Check sheet for the drawn part. Datum: minimum x, y, z corner. Units: mm. Give positions to 0.01 mm unless a question says otherwise; leave off trailing zeros. Order: outer loops, then holes, each group sorted by start corner. A loop starts at its lowest first (then second) coordinate and runs counter-clockwise, first axis right, second up. Notation, with made-up numbers: (15, 56.25) -> (53, 56.25) arc R13 cw to (53, 76.25) -> close; hole circle Ø3 at (-25.75, -28). An arc over 180 degrees is marked (long way). Return JSON: item names as keys, results as strings. Group by question number.
(1) Cross-section at A-A on z = 3.45. Enter the section's corners in (x, y).
(2) Cross-section at B-B on x = 15.25. Enter the section's corners in (y, z) (3 decimals), then the cut area to 3 significant figures.
(3) Cross-section at C-C on y = 95. Enter the section's corners in (x, z), then the cut area to 3 significant figures.
(4) Thickness scan on line 1 along X through (y, z) = (53.5, 3.8); line 2 along X through (y, z) = (51, 1.2); line 3 along Y through (x, z) = (3.25, 3.15). Record the ranges inside material, lowest first.
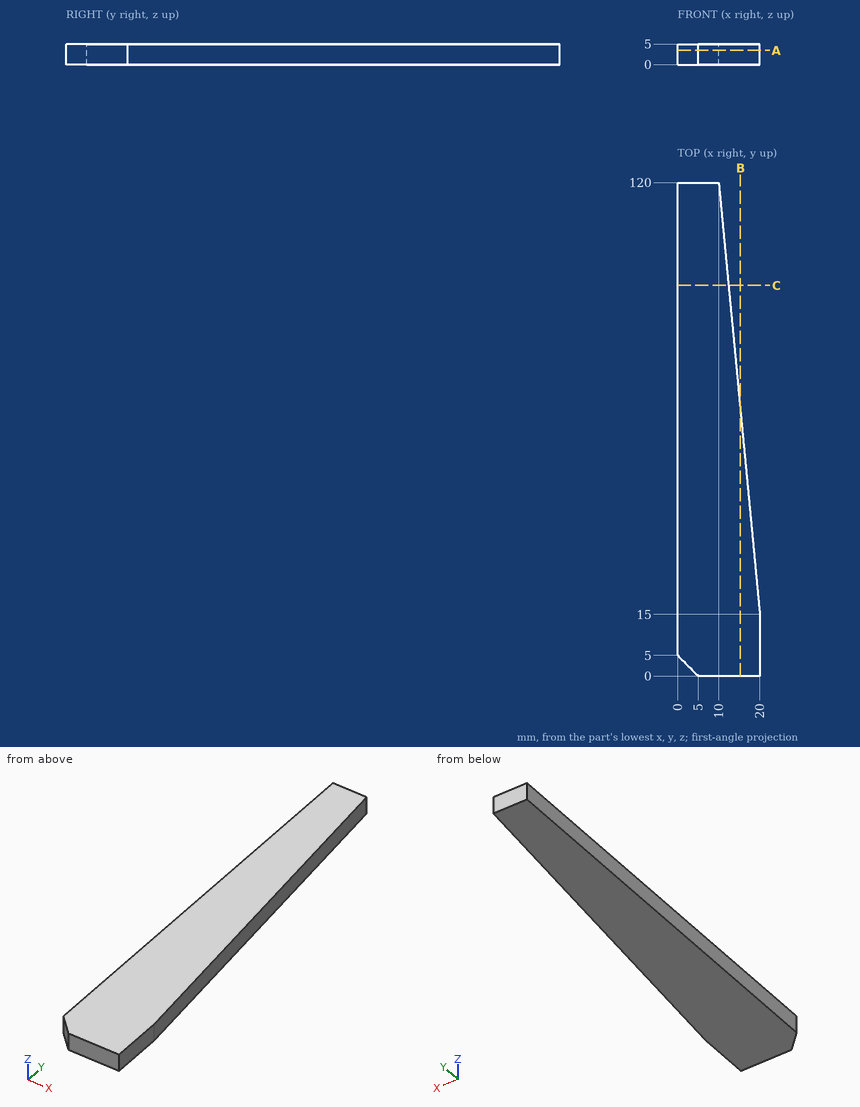
Verdict:
{
 "1": {"outline": "(0, 5) -> (5, 0) -> (20, 0) -> (20, 15) -> (10, 120) -> (0, 120) -> close"},
 "2": {"outline": "(0, 0) -> (64.875, 0) -> (64.875, 5) -> (0, 5) -> close", "area": "324 mm²"},
 "3": {"outline": "(0, 0) -> (12.38, 0) -> (12.38, 5) -> (0, 5) -> close", "area": "61.9 mm²"},
 "4": {"line 1": "0 to 16.33", "line 2": "0 to 16.57", "line 3": "1.75 to 120"}
}
